Geometry: final body of the model. Coordinates: model frame, mm. A direction names the side the tool comes from. Round coordinates to 2 decimals unless told otherwise and drop trailing zeros. Write each loop counter-clockwise with the first axis right and the second up, starting at its lowest first coordinate (ties: lowest second). Pieces come first, ordered by that corner, then holes. Notation, with made-up numbers: M 80.5,20.5 L 118.5,20.5 A20 ccw 118.5,32.5 Z; hole C 43.25,44.25 d8. An arc over 180 degrees is marked long. Put each result on its own line as item: value. Start each with the question number.
```python
from build123d import *

# Parameters (mm, degrees)
SKETCH1_R           = 5
BOSS_EXTRUDE1_DEPTH = 65
CHAMFER1_SIZE       = 0.5


with BuildPart() as part:
    # Sketch1 → Boss-Extrude1 (new body)
    with BuildSketch(Plane(origin=(0, 0, 0), x_dir=(1, 0, 0), z_dir=(0, 1, 0))):
        with Locations(Location((0, 0, 0), (0, 0, 270))):
            Circle(SKETCH1_R)
    extrude(amount=BOSS_EXTRUDE1_DEPTH)

    # Sketch2 → Ø18.0 (18) Diameter Hole1 (revolve, cut)
    with BuildSketch(Plane(origin=(0, 65, 0), x_dir=(0, 0, 1), z_dir=(1, 0, 0))):
        Polygon((0, 0), (0, 11.802581857), (3, 10), (3, 0), align=None)
    f_18_0_18_diameter_hole1 = revolve(axis=Axis((0, 71.35, 0), (0, -1, 0)), mode=Mode.SUBTRACT)

    # Mirror1: Ø18.0 (18) Diameter Hole1 across plane
    add(f_18_0_18_diameter_hole1.mirror(Plane.ZX.offset(32.5)), mode=Mode.SUBTRACT)

    # Chamfer1
    chamfer1_edges = [part.edges().sort_by_distance(p)[0] for p in [
        (0, 0, -5),
        (0, 65, -5),
    ]]
    chamfer(chamfer1_edges, length=CHAMFER1_SIZE)


solid = part.part
```
1) Section A-A, the plane y = 32.5. Output: boundary loops of the cut face in (x, z), and give its area (3 significant figures).
2) First-contact query: pin 1 (1 mm diameter, centred on x = 0.5, z = -2.5, fed in from +Y); pin 2 (1 mm diameter, centred on x = 2, y = 17, fed in from -Z); pin 3 (3.5 mm diameter, centred on x = 0, z = 0, fed in from -Y); pin 4 (1.5 mm diameter, centred on y = 34.5, z = -1.5, fed in from -X). Flat tips, straight axial feed; report the tip coordinate or a pass-through.
3) Access query for faces 4 (the face through (0.51, 53.51, -0.11)), 5 (the face through (0, 5, -3)). Directions: +Z, -Z, +X, -X, +Y, -Y. A direction counts if a zero-diameter tool reaches every point of the face in a straight line with its end or side. Return the directions, or none.
4) Ray query, probe 1 along X at (y, z) = (2.25, 0); probe 2 along X at (y, z) = (59.5, -4); probe 3 along X at (y, z) = (49.5, -2.25). Return the intervals inside material, ascending.
5) Draft query along Z for faces 1 (the face through (-3, 65, 1)), 2 (the face through (-4.88, 32.05, -1.08)), 3 (the face through (0, 60, -3)). Return one class per face: +Z half, -Z half, draft (parallel to the pull), parting line (faces both ways), or undercut.
Solved:
1. outline: C 0,0 d10
1. area: 78.5 mm2
2. pin 1: stops at y = 65
2. pin 2: stops at z = -4.77
2. pin 3: stops at y = 10.75
2. pin 4: stops at x = -4.94
3. face 4: +Y
3. face 5: -Y
4. probe 1: x = -5 to -3, 3 to 5
4. probe 2: x = -3 to 3
4. probe 3: x = -4.47 to 4.47
5. face 1: draft
5. face 2: parting line
5. face 3: undercut
